For this review, use the dimensioned drawing (mm, ordinates from the lowest corner) and the shaded views. A direction names the side the tool comes from. Round coordinates to 2 decimals unless told otherwise and drop trailing zeros. Loops run counter-clockwise (first coordinate to the right, second up) from the corner with the lowest first, then second, coordinate; pieces in that order, holes last. Notation, with made-up numbers: M 10,74 L 37,74 A14 cw 37,94 Z; hole C 6.5,24 d7. An arc over 180 degrees is marked long. Answer as a JSON object with one key per item and string values. Group by question number.
Item 1: Consider section A-A (z = 4.75). Give the boundary of the cut face in (x, y), and give its area (3 significant figures).
Item 2: The part is to be moulded in two halves that separate along Y. For the marked faces 1, 2, 3 and 4, say which applies: +Y half, -Y half, draft (parallel to the pull), parting line (faces both ways), or undercut.
Item 3: Tool access review of the marked faces 5 and 6: name each direction out of +Z, -Z, +X, -X, +Y, -Y from which nothing blocks a thin tool from reaching the whole face with its end or side.
Item 4: Insertion check: P1, Ø3, axis at x = 4, y = 3, coming from the +Z side; P2, Ø1.5, axis at y = 3.5, z = 13, coming from the -X side. Each pin has a flat end and moves straight along its axis. Give the tip position at first contact, or say it passes through.
Item 5: To check wall thickness, follow line 1 (Z direction, x = 8.25, y = 8); line 2 (Z direction, x = 3.5, y = 6.75); line 3 (X direction, y = 2.25, z = 8.5) (1 decimal). State the ranges of each line that lie inside material, in increasing order.
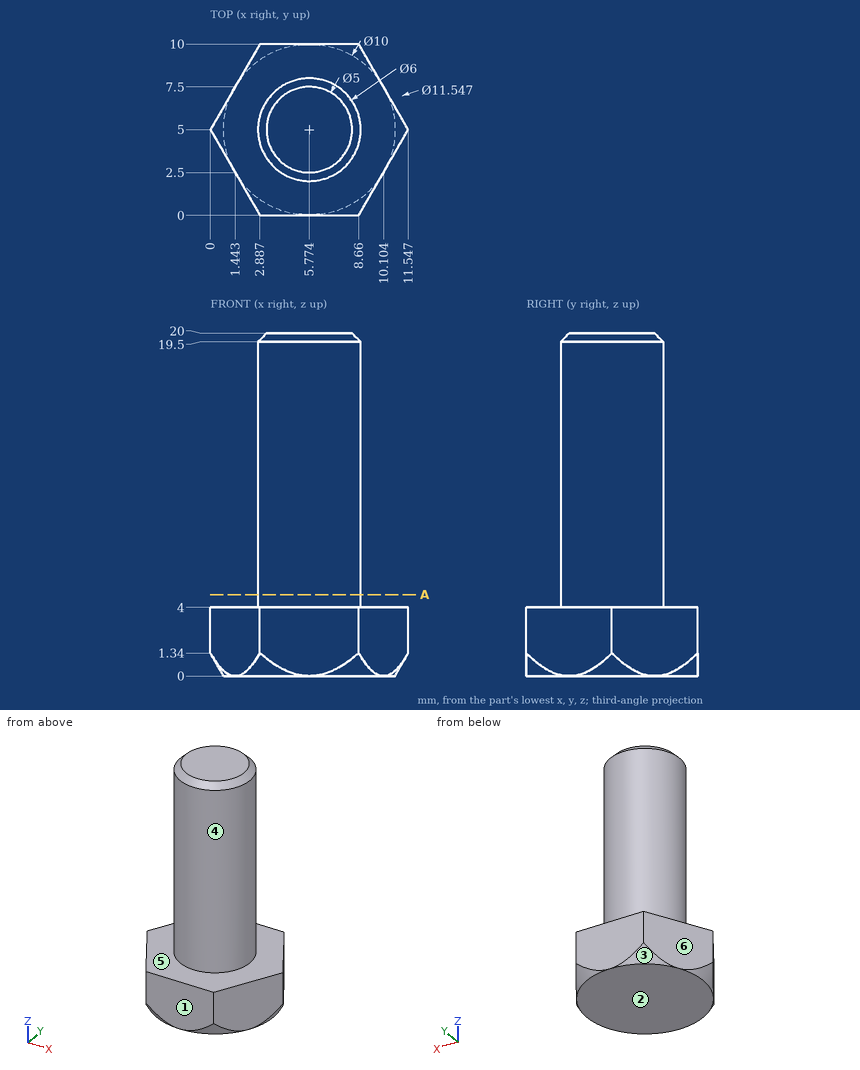
Geometry results:
{
 "1": {"outline": "C 5.77,5 d6", "area": "28.3 mm^2"},
 "2": {"face 1": "-Y half", "face 2": "draft", "face 3": "+Y half", "face 4": "parting line"},
 "3": {"face 5": "+Z", "face 6": "+Z, -Z, -X, +Y"},
 "4": {"P1": "stops at z = 20", "P2": "stops at x = 2.87"},
 "5": {"line 1": "z = 0 to 4", "line 2": "z = 0 to 19.63", "line 3": "x = 4.6 to 7"}
}
